Source: CAD feature listing. Evaluate the final solid. Frame: model axes, mm. A direction names the side the tool comes from. Round coordinates to 2 decimals unless told otherwise and drop trailing zeros. Order: outer loops, then holes, each group sorted by start corner. A loop starts at its lowest first (then second) coordinate and runs counter-clockwise, first axis right, second up. Notation, with made-up numbers: (31.5, -23.5) -> (71.5, -23.5) arc R19 ccw to (71.5, -0.5) -> close; hole circle Ø3 at (45.25, 44). An arc over 180 degrees is marked (long way). One line per item, written item: value. Start each with the question number.
1) Section D-D (x = 8). Return the cut outline in (y, z), and give its area (3 significant figures).
2) Reachability of faces 1 (the face through (10.5, 0.1, -11.9)), 2 (the face through (0, 0, 54)), 3 (the face through (-6, -3, 0)) from +Z, -Z, +X, -X, +Y, -Y: full face, straight path, thin tool, end or side. Return the list, or none.
3) Section C-C (z = -11). Return the cut outline in (x, y), and give its area (3 significant figures).
4) Section A-A (y = 0). Return the cut outline in (x, z).
5) Pin query (flat end, axial travel): P1, Ø12, axis at x = -5, y = 1.5, coming from the -Z side; P2, Ø1.5, axis at x = -9, y = 3.5, coming from the +Z side; P3, Ø10, axis at y = 5.5, z = 44.5, coming from the +X side. Return the tip coordinate at first contact, or that it passes through.
6) Section B-B (x = 0). Return the cut outline in (y, z).
7) Ray query, L1, parallel to Z at x = -8.5, y = -6; L2, parallel to Y at x = 8, z = -8.5; L3, parallel to X at y = 2.25, z = 24. Return the intervals inside material, ascending.
```python
from build123d import *

# Parameters (mm, degrees)
MAIN_JOURNAL_PROFILE_12_R = 6
MAIN_JOURNAL_12_DEPTH     = 30
STEP_JOURNAL_PROFILE_9_R  = 4.5
STEP_JOURNAL_9_DEPTH      = 12
SHAFT_END_PROFILE_5_R     = 2.5
SHAFT_END_5_DEPTH         = 12
CRANK_WEB_DEPTH           = 8
CRANK_PIN_PROFILE_R       = 2.5
CRANK_PIN_DEPTH           = 8


with BuildPart() as part:
    # Main Journal Profile Ø12 → Main Journal Ø12 (new body)
    with BuildSketch(Plane.XY):
        Circle(MAIN_JOURNAL_PROFILE_12_R)
    extrude(amount=MAIN_JOURNAL_12_DEPTH)

    # Step Journal Profile Ø9 → Step Journal Ø9 (add)
    with BuildSketch(Plane.XY.offset(30)):
        Circle(STEP_JOURNAL_PROFILE_9_R)
    extrude(amount=STEP_JOURNAL_9_DEPTH)

    # Shaft End Profile Ø5 → Shaft End Ø5 (add)
    with BuildSketch(Plane.XY.offset(42)):
        Circle(SHAFT_END_PROFILE_5_R)
    extrude(amount=SHAFT_END_5_DEPTH)

    # Crank Web Profile → Crank Web (add)
    with BuildSketch(Plane(origin=(0, 0, 0), x_dir=(-1, 0, 0), z_dir=(0, 0, -1))):
        with BuildLine():
            ThreePointArc((-12.779377919, 3.5), (-13.25, 0), (-12.779377919, -3.5))
            ThreePointArc((-12.779377919, -3.5), (-3.699194839, -6.657412557), (3.777827997, -12.7000203))
            ThreePointArc((3.777827997, -12.7000203), (13.25, 0), (3.777827997, 12.7000203))
            ThreePointArc((3.777827997, 12.7000203), (-3.699194839, 6.657412557), (-12.779377919, 3.5))
        make_face()
    extrude(amount=CRANK_WEB_DEPTH)

    # Crank Pin Profile → Crank Pin (add)
    with BuildSketch(Plane(origin=(0, 0, -8), x_dir=(-1, 0, 0), z_dir=(0, 0, -1))):
        with Locations((-8, 0)):
            Circle(CRANK_PIN_PROFILE_R)
    extrude(amount=CRANK_PIN_DEPTH)


solid = part.part
```
Findings:
1. outline: (-4.72, -8) -> (-2.5, -8) -> (-2.5, -16) -> (2.5, -16) -> (2.5, -8) -> (4.72, -8) -> (4.72, 0) -> (-4.72, 0) -> close
1. area: 116 mm2
2. face 1: -Z
2. face 2: +Z, +X, -X, +Y, -Y
2. face 3: +Z
3. outline: circle Ø5 at (8, 0)
3. area: 19.6 mm2
4. outline: (-13.25, -8) -> (5.5, -8) -> (5.5, -16) -> (10.5, -16) -> (10.5, -8) -> (13.25, -8) -> (13.25, 0) -> (6, 0) -> (6, 30) -> (4.5, 30) -> (4.5, 42) -> (2.5, 42) -> (2.5, 54) -> (-2.5, 54) -> (-2.5, 42) -> (-4.5, 42) -> (-4.5, 30) -> (-6, 30) -> (-6, 0) -> (-13.25, 0) -> close
5. P1: z = -8
5. P2: z = 0
5. P3: x = 4.35
6. outline: (-9.12, -8) -> (9.12, -8) -> (9.12, 0) -> (6, 0) -> (6, 30) -> (4.5, 30) -> (4.5, 42) -> (2.5, 42) -> (2.5, 54) -> (-2.5, 54) -> (-2.5, 42) -> (-4.5, 42) -> (-4.5, 30) -> (-6, 30) -> (-6, 0) -> (-9.12, 0) -> close
7. L1: -8 to 0
7. L2: -2.5 to 2.5
7. L3: -5.56 to 5.56
